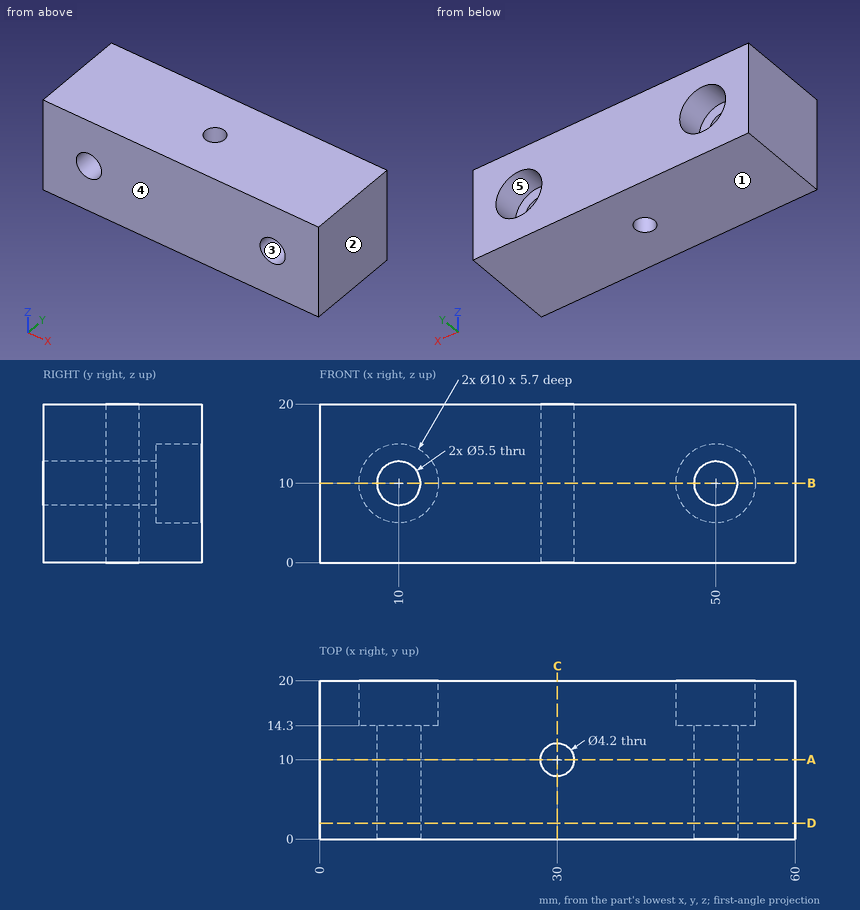
Geometry check sheet. Reference: drawing and pictorial views, mm from the part's lowest x, y, z. A direction names the side the tool comes from. Round coordinates to 2 decimals unless told otherwise and drop trailing zeros. Loops run counter-clockwise (first coordinate to the right, second up) from the corner with the lowest first, then second, coordinate; pieces in that order, holes last. Notation, with made-up numbers: (-39, -4.75) -> (-33, -4.75) arc R23 cw to (-33, 33.25) -> close; hole circle Ø9 at (-38, 78.5). An arc over 180 degrees is marked (long way). Answer as a JSON object with one key per item and string values.
Q1. Access from +Z, -Z, +X, -X, +Y, -Y to the whole of each face (thin tool, end or side, straight path). Record for the marked faces 4 and 5.
Data:
{"face 4": "+Z, -Z, +X, -X, -Y", "face 5": "+Y"}
Q2. Draft check along X on the marked faces 1, 2 and 3. Enter one of: pulls with the +X half, pulls with the -X half, needs draft (parallel to the pull), parting line crosses it, or undercut.
Data:
{"face 1": "needs draft", "face 2": "pulls with the +X half", "face 3": "undercut"}
Q3. Scan lines: line 1 (X direction, y = 1, z = 9); line 2 (Z direction, x = 50, y = 18.65); line 3 (Z direction, x = 50, y = 4). Record each from-to range of solid material in increasing order. Write a range as from..to.
Data:
{"line 1": "x = 0..7.44, 12.56..47.44, 52.56..60", "line 2": "z = 0..5, 15..20", "line 3": "z = 0..7.25, 12.75..20"}
Q4. Section check A-A (y = 10). Record the boundary of the cut face in (x, z).
Data:
{"outline": "(0, 0) -> (27.9, 0) -> (27.9, 20) -> (0, 20) -> close; (32.1, 0) -> (60, 0) -> (60, 20) -> (32.1, 20) -> close; hole circle Ø5.5 at (10, 10); hole circle Ø5.5 at (50, 10)"}
Q5. Section check C-C (x = 30). Record the boundary of the cut face in (y, z), then the cut area to 3 significant figures.
Data:
{"outline": "(0, 0) -> (7.9, 0) -> (7.9, 20) -> (0, 20) -> close; (12.1, 0) -> (20, 0) -> (20, 20) -> (12.1, 20) -> close", "area": "316 mm2"}
Q6. Section check B-B (z = 10). Record the boundary of the cut face in (x, y), then the cut area to 3 significant figures.
Data:
{"outline": "(0, 0) -> (7.25, 0) -> (7.25, 14.3) -> (5, 14.3) -> (5, 20) -> (0, 20) -> close; (12.75, 0) -> (47.25, 0) -> (47.25, 14.3) -> (45, 14.3) -> (45, 20) -> (15, 20) -> (15, 14.3) -> (12.75, 14.3) -> close; (52.75, 0) -> (60, 0) -> (60, 20) -> (55, 20) -> (55, 14.3) -> (52.75, 14.3) -> close; hole circle Ø4.2 at (30, 10)", "area": "915 mm2"}
Q7. Go/stop test with a flat-tipped pin: P1, Ø3, axis at x = 50, z = 8.5, coming from the +Y side. Record where the tip stops, or that it passes through.
Data:
{"P1": "stops at y = 14.3"}
Q8. Section check D-D (y = 2). Record the boundary of the cut face in (x, z).
Data:
{"outline": "(0, 0) -> (60, 0) -> (60, 20) -> (0, 20) -> close; hole circle Ø5.5 at (10, 10); hole circle Ø5.5 at (50, 10)"}
